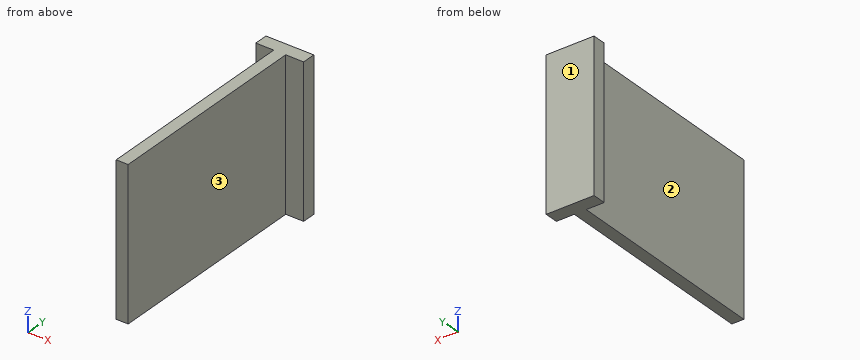
```python
from build123d import *

# Parameters (mm, degrees)
EXTRUDE_1_DEPTH = 100


with BuildPart() as part:
    # 草图1 → 凸台-拉伸1 (new body)
    with BuildSketch(Plane.XY):
        Polygon((-32.039764657, -6.511895803), (-32.039764657, -120.09527648), (-32.039764657, -146.511895803), (-24.039764657, -146.511895803), (-24.039764657, -120.09527648), (-24.039764657, -6.511895803), (-12.039764657, -6.511895803), (-12.039764657, 2.488104197), (-44.039764657, 2.488104197), (-44.039764657, -6.511895803), align=None)
    extrude(amount=EXTRUDE_1_DEPTH)


solid = part.part
```
Geometry check sheet. Reference: the model listing, model coordinates, mm. Face numbers are marked on the shaded views. A direction names the side the tool comes from. Coordinates: 2 decimals unless noted, no trailing zeros. Loops run counter-clockwise (first coordinate to the right, second up) from the corner with the lowest first, then second, coordinate; pieces in that order, holes last.
Item 1: Go/stop test with flat-tipped pins: pin 1 Ø12 at (y, z) = (-43, 55.5) entering from -X; pin 2 Ø5 at (x, y) = (-35, -47.5) entering from +Z; pin 3 Ø3.5 at (x, z) = (-37, 61) entering from -Y; pin 4 Ø4 at (x, y) = (-22.5, -25) entering from -Z. Record where each tip stops, or that it passes through.
Item 2: Sectioned sample at A-A, the plane z = 47. Record the boundary of the cut face in (x, y).
Item 3: Sectioned sample at C-C, the plane x = -35.5. Record the boundary of the cut face in (y, z), then the cut area to 3 significant figures.
Item 4: Sectioned sample at B-B, the plane y = -14. Record the boundary of the cut face in (x, z).
Item 5: Access from +Z, -Z, +X, -X, +Y, -Y to the whole of each face (thin tool, end or side, straight path). Record for the marked faces 1, 2 and 3.
Item 6: Thickness scan on line 1 (X direction, y = -132.5, z = 96); line 2 (Y direction, x = -36, z = 51.5). Record the ranges inside material, lowest first.
Check result:
1. pin 1: stops at x = -32.04
1. pin 2: passes through
1. pin 3: stops at y = -6.51
1. pin 4: stops at z = 0
2. outline: (-44.04, -6.51) - (-32.04, -6.51) - (-32.04, -146.51) - (-24.04, -146.51) - (-24.04, -6.51) - (-12.04, -6.51) - (-12.04, 2.49) - (-44.04, 2.49) - close
3. outline: (-6.51, 0) - (2.49, 0) - (2.49, 100) - (-6.51, 100) - close
3. area: 900 mm2
4. outline: (-32.04, 0) - (-24.04, 0) - (-24.04, 100) - (-32.04, 100) - close
5. face 1: +Z, -Z, +X, -X, +Y
5. face 2: +Z, -Z, -X, -Y
5. face 3: +Z, -Z, +X, -Y
6. line 1: x = -32.04 to -24.04
6. line 2: y = -6.51 to 2.49
